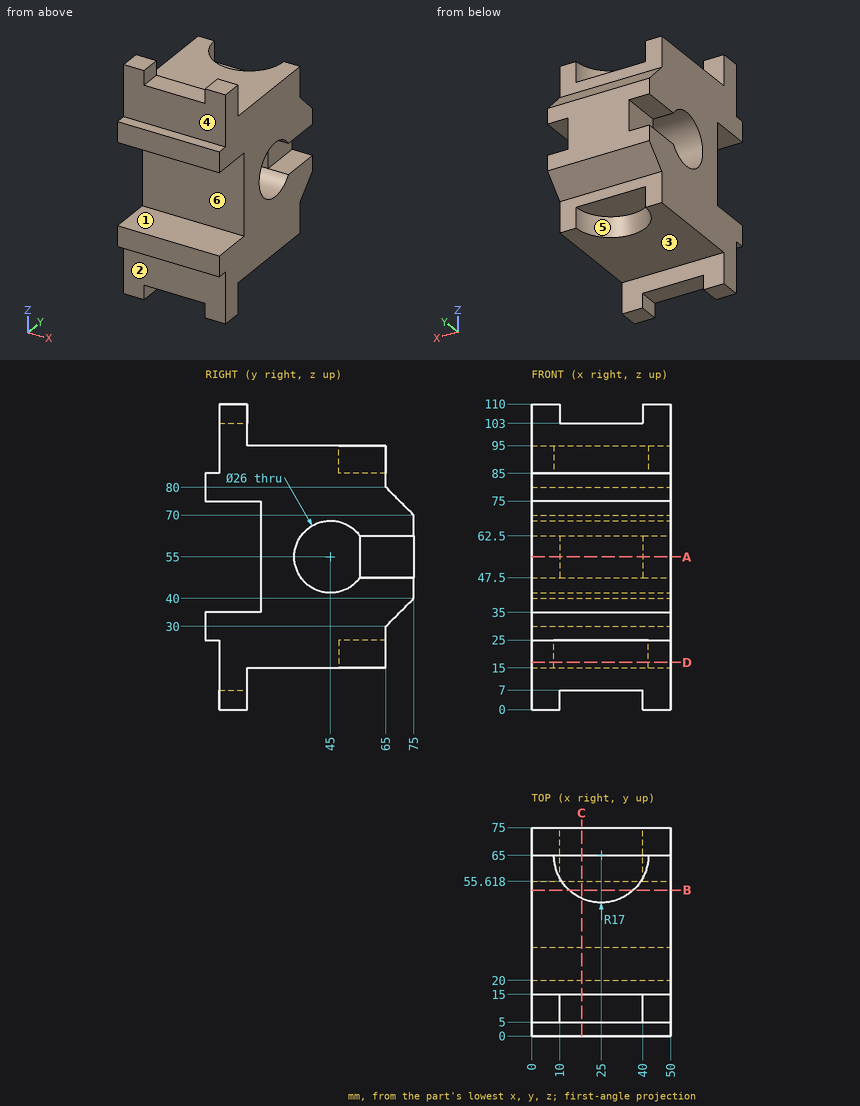
Study the drawing (mm; zero at the part's minimum x, y, z) and answer. A direction names the side the tool comes from. Coordinates: 2 decimals unless noted, no trailing zeros. Write each loop counter-clockwise with the first axis right and the second up, starting at its lowest first coordinate (ties: lowest second). Pieces come first, ordered by that corner, then holes. Notation, with made-up numbers: (10.5, 77) - (18.5, 77) arc R19 ccw to (18.5, 101) - close; hole circle Ø1 at (31, -1). An arc over 180 degrees is marked (long way). Answer as a JSON object with one key per item and string values.
Q1. Find section B-B (y = 52.5). Write down the section's boundary in (x, z).
Results list:
{"outline": "(0, 15) - (13.48, 15) - (13.48, 25) - (36.52, 25) - (36.52, 15) - (50, 15) - (50, 44.38) - (0, 44.38) - close; (0, 65.62) - (50, 65.62) - (50, 95) - (36.52, 95) - (36.52, 85) - (13.48, 85) - (13.48, 95) - (0, 95) - close"}
Q2. Consider L1, parallel to Y at x = 16.5, z = 55; L2, parallel to Z at x = 17.5, y = 19; L3, parallel to Z at x = 33.5, y = 26.5. Determine where each line is inside the solid, lowest interval first. Write a range as from..to.
Results list:
{"L1": "y = 20..32, 55.62..75", "L2": "z = 15..35, 75..95", "L3": "z = 15..95"}
Q3. Find section C-C (x = 18). Write down the section's boundary in (y, z).
Results list:
{"outline": "(0, 25) - (5, 25) - (5, 7) - (15, 7) - (15, 15) - (49.51, 15) - (49.51, 25) - (65, 25) - (65, 30) - (75, 40) - (75, 70) - (65, 80) - (65, 85) - (49.51, 85) - (49.51, 95) - (15, 95) - (15, 103) - (5, 103) - (5, 85) - (0, 85) - (0, 75) - (20, 75) - (20, 35) - (0, 35) - close; hole (55.62, 47.5) - (55.62, 62.5) arc R13 ccw (long way) to start"}
Q4. Given pin 1 Ø3 at (x, y) = (45.5, 63.5) entering from +Z; pin 2 Ø16.5 at (x, z) = (34.5, 24) entering from +Y; pin 3 Ø20 at (x, z) = (15.5, 45.5) entering from -Y; pin 4 Ø2 at (y, z) = (34, 55.5) entering from +X, each flat-ended and moving along its own axis, determine where each tip first touches the part or whether it passes through.
Results list:
{"pin 1": "stops at z = 95", "pin 2": "stops at y = 67.25", "pin 3": "stops at y = 20", "pin 4": "passes through"}
Q5. Which of the six approach directions +Z, -Z, +X, -X, +Y, -Y give full straight-line access (tool end or side, diameter ignored) to the marked faces 4, 5 and 6?
Results list:
{"face 4": "+Z, +X, -X, -Y", "face 5": "-Z, +Y", "face 6": "+X, -X, -Y"}
Q6. Find section A-A (z = 55). Write down the section's boundary in (x, y), plus the area to 3 significant figures.
Results list:
{"outline": "(0, 20) - (50, 20) - (50, 32) - (0, 32) - close; (10, 55.62) - (40, 55.62) - (40, 75) - (10, 75) - close", "area": "1,180 mm^2"}
Q7. Find section D-D (z = 17). Write down the section's boundary in (x, y), plus the area to 3 significant figures.
Results list:
{"outline": "(0, 5) - (50, 5) - (50, 65) - (42, 65) arc R17 cw to (8, 65) - (0, 65) - close", "area": "2,550 mm^2"}
Q8. For a pull along Z with two mould halves and no side action, classify the marked faces 1, 2 and 3 as pulls with the +Z half, pulls with the -Z half, needs draft (parallel to the pull), parting line crosses it, or undercut.
Results list:
{"face 1": "undercut", "face 2": "needs draft", "face 3": "pulls with the -Z half"}
